from build123d import *

# Parameters (mm, degrees)
SKETCH_1_W          = 63
SKETCH_1_H          = 24
SKETCH_1_W_2        = 50
SKETCH_1_H_2        = 18
SKETCH_5_R          = 2.25
CUT_EXTRUDE_3_DEPTH = 334.514992167


with BuildPart() as part:
    # 扫描1: sweep along a path in 草图2
    with BuildLine(Plane(origin=(0, 0, 0), x_dir=(0, 0, -1), z_dir=(1, 0, 0))) as sweep_1_path:
        Line((0, 0), (134, 0))
        ThreePointArc((134, 0), (184, 50), (134, 100))
        Line((134, 100), (-308, 100))
    # 草图1 → 扫描1 (sweep)
    with BuildSketch(Plane.XY):
        Rectangle(SKETCH_1_W, SKETCH_1_H)
        Rectangle(SKETCH_1_W_2, SKETCH_1_H_2, mode=Mode.SUBTRACT)
    sweep(path=sweep_1_path.line)

    # 草图5 → 切除-拉伸3 (cut, through all)
    with BuildSketch(Plane.XZ.offset(12)):
        with Locations((-17.5, -10)):
            Circle(SKETCH_5_R)
        with Locations((17.5, -10)):
            Circle(SKETCH_5_R)
        with Locations(Location((-17.5, 298, 0), (0, 0, 180))):
            Circle(SKETCH_5_R)
        with Locations(Location((17.5, 298, 0), (0, 0, 180))):
            Circle(SKETCH_5_R)
    extrude(amount=-CUT_EXTRUDE_3_DEPTH, mode=Mode.SUBTRACT)


solid = part.part
Geometry: final body of the model. Coordinates: model frame, mm. A direction names the side the tool comes from. Give positions to 0.01 mm unless a question says otherwise; leave off trailing zeros. Loops run counter-clockwise (first coordinate to the right, second up) from the corner with the lowest first, then second, coordinate; pieces in that order, holes last. Notation, with made-up numbers: M 64.5,83.5 L 119.5,83.5 A19 ccw 119.5,105.5 Z; hole C 64,45 d3. An arc over 180 degrees is marked long. Put each result on its own line as item: value. Start each with the question number.
1) Ray query, line 1 along Y through (x, z) = (12.5, -130); line 2 along X through (y, z) = (90, 298); line 3 along X through (y, z) = (-5, -140). Return the intervals inside material, ascending.
2) Cut plane C-C (y = 50). Output: boundary loops of the cut face in (x, z).
3) Cut plane A-A (z = -107). Output: boundary loops of the cut face in (x, y), then the cut area to 3 significant figures.
4) Access query for faces 4 (the flat face through (-25, 98, 1)), 5 (the cylindrical face through (0.441, 48.637, -195.985)), 6 (the flat face through (0, 91, 90)), 7 (the flat face through (0, 12, -68)), 8 (the flat face through (0, -10, 0)). Directions: +Z, -Z, +X, -X, +Y, -Y. A direction counts if a zero-diameter tool reaches every point of the face in a straight line with its end or side. Return the directions, or none.
5) Cut plane B-B (x = 9). Output: boundary loops of the cut face in (y, z).
6) Pull-direction query (Y, two-part tool) for faces 1 (the flat face through (0, 112, 90)), 2 (the flat face through (-31.5, 92, 17)), 3 (the flat face through (0, 9, -68)); classes: pulls with the +Y half, pulls with the -Y half, needs draft (parallel to the pull), parting line crosses it, or undercut.
7) Cut plane D-D (z = 239). Output: boundary loops of the cut face in (x, y).
8) Contact query for flat-ended pins moving along their axis: pin 1 (1 mm diameter, centred on x = 14.5, y = 75.5, fed in from +Z); pin 2 (6 mm diameter, centred on x = -15, y = 95, fed in from -Z); pin 3 (6 mm diameter, centred on x = -17.5, z = 298, fed in from -Y); pin 4 (6 mm diameter, centred on x = -17.5, z = -10, fed in from -Y). Output: stop coordinate, or through.
Verdict:
1. line 1: -12 to -9, 9 to 12, 88 to 91, 109 to 112
1. line 2: -31.5 to -19.75, -15.25 to 15.25, 19.75 to 31.5
1. line 3: -31.5 to -25, 25 to 31.5
2. outline: M -31.5,-196 L 31.5,-196 L 31.5,-172 L -31.5,-172 Z; hole M -25,-193 L 25,-193 L 25,-175 L -25,-175 Z
3. outline: M -31.5,-12 L 31.5,-12 L 31.5,12 L -31.5,12 Z; M -31.5,88 L 31.5,88 L 31.5,112 L -31.5,112 Z; hole M -25,-9 L 25,-9 L 25,9 L -25,9 Z; hole M -25,91 L 25,91 L 25,109 L -25,109 Z
3. area: 1,220 mm2
4. face 4: none
4. face 5: -Z, +X, -X
4. face 6: +Z
4. face 7: +Z, +X, -X
4. face 8: +Z, +X, -X, -Y
5. outline: M -12,-134 A62 ccw 112,-134 L 112,308 L 109,308 L 109,-134 A59 cw -9,-134 L -9,0 L -12,0 Z; M 9,-134 A41 ccw 91,-134 L 91,308 L 88,308 L 88,-134 A38 cw 12,-134 L 12,0 L 9,0 Z
6. face 1: pulls with the +Y half
6. face 2: needs draft
6. face 3: undercut
7. outline: M -31.5,88 L 31.5,88 L 31.5,112 L -31.5,112 Z; hole M -25,91 L 25,91 L 25,109 L -25,109 Z
8. pin 1: z = -161.71
8. pin 2: z = -179.61
8. pin 3: y = 88
8. pin 4: y = -12
